CAD build for the part. Positions are in the model's coordinates, mm. Coordinates: 2 decimals unless noted, no trailing zeros. Write each loop counter-clockwise with the first axis right and the second up, starting at its lowest first coordinate (ties: lowest second). Pieces come first, ordered by that corner, then holes. Notation, with made-up numbers: M 67.5,3 L 106.5,3 A24 cw 106.5,24 Z; hole C -23,5 d4. An arc over 180 degrees is marked long. Put each result on its own line as item: value. Start each with the question number.
```python
from build123d import *

# Parameters (mm, degrees)
EXTRUDE_1_DEPTH           = 250
HOLE_WIZARD_1_D           = 3.4
HOLE_WIZARD_1_CBORE_D     = 6
HOLE_WIZARD_1_CBORE_DEPTH = 3.4


with BuildPart() as part:
    # 草圖1 → 伸長1 (new body)
    with BuildSketch(Plane.XY):
        Polygon((-3, 4.5), (3, 4.5), (3, -4.5), (-3, -4.5), (-3, -1.7), (-1.5, -1.7), (-1.5, -2.85), (1.5, -2.85), (1.5, 2.85), (-1.5, 2.85), (-1.5, 1.7), (-3, 1.7), align=None)
    extrude(amount=EXTRUDE_1_DEPTH)

    # 打孔尺寸(%根据)内六角圆柱头螺钉的类型1 (through all)
    with Locations(Plane.ZY.offset(3)):
        with Locations((245, 0), (5, 0)):
            CounterBoreHole(HOLE_WIZARD_1_D / 2, HOLE_WIZARD_1_CBORE_D / 2, HOLE_WIZARD_1_CBORE_DEPTH)


solid = part.part
```
(1) Two-plate mould, pull along Y, no slides. Class faces 1 (the face through (1.5, 0, 123)), 2 (the face through (2, 0, 250)), 3 (the face through (0, 4.5, 123)), 4 (the face through (0, -4.5, 123)): +Y half, -Y half, draft (parallel to the pull), parting line (faces both ways), or undercut.
(2) Drop a flat-ended pin along its axis: pin 1 (4 mm diameter, centred on y = -1.5, z = 163, fed in from -X). Give the stop position or say it passes through.
(3) Slice it at A-A, the plane y = 0. Write the cut outline in (x, z), then the cut area to 3 significant figures.
(4) Drill centre lines: line 1 (Z direction, x = -2.4, y = 2.5); line 2 (X direction, y = 2.75, z = 106.5); line 3 (Y direction, x = 0.05, z = 188). Where is each one in solid material? Low to high. Write a range as [from, to].
(5) Slice it at B-B, the plane z = 169. Write the cut outline in (x, y).
Result set:
1. face 1: undercut
1. face 2: draft
1. face 3: +Y half
1. face 4: -Y half
2. pin 1: stops at x = -3
3. outline: M 1.5,0 L 3,0 L 3,3.3 L 1.5,3.3 Z; M 1.5,6.7 L 3,6.7 L 3,243.3 L 1.5,243.3 Z; M 1.5,246.7 L 3,246.7 L 3,250 L 1.5,250 Z
3. area: 365 mm^2
4. line 1: z = [0, 3.34], [6.66, 243.34], [246.66, 250]
4. line 2: x = [-3, -1.5], [1.5, 3]
4. line 3: y = [-4.5, -2.85], [2.85, 4.5]
5. outline: M -3,-4.5 L 3,-4.5 L 3,4.5 L -3,4.5 L -3,1.7 L -1.5,1.7 L -1.5,2.85 L 1.5,2.85 L 1.5,-2.85 L -1.5,-2.85 L -1.5,-1.7 L -3,-1.7 Z
